The model under review builds one solid part; all positions refer to its coordinate system, in mm. Coordinates: 2 decimals unless noted, no trailing zeros. Write each loop counter-clockwise with the first axis right and the second up, starting at its lowest first coordinate (ties: lowest second). Pieces come first, ordered by that corner, then holes. Notation, with made-up numbers: (41.25, -6) - (77.25, -6) arc R17 ccw to (77.25, 12) - close; hole circle Ø4 at (0.25, 54). An arc over 180 degrees is marked (long way). Put each result on its own line as item: value.
from build123d import *

# Parameters (mm, degrees)
SKETCH_1_W          = 80
SKETCH_1_H          = 90
EXTRUDE_1_DEPTH     = 3
SKETCH_2_R          = 4.5
SKETCH_2_R_2        = 8.1
CUT_EXTRUDE_1_DEPTH = 13


with BuildPart() as part:
    # 草图1 → 凸台-拉伸1 (new, symmetric)
    with BuildSketch(Plane.XY):
        Rectangle(SKETCH_1_W, SKETCH_1_H)
    extrude(amount=EXTRUDE_1_DEPTH, both=True)

    # 草图2 → 切除-拉伸1 (cut, symmetric)
    with BuildSketch(Plane.XY):
        with Locations((-30, -30)):
            Circle(SKETCH_2_R)
        with Locations((-30, 30)):
            Circle(SKETCH_2_R)
        with Locations((30, -30)):
            Circle(SKETCH_2_R)
        with Locations((30, 30)):
            Circle(SKETCH_2_R)
        Circle(SKETCH_2_R_2)
    extrude(amount=CUT_EXTRUDE_1_DEPTH, both=True, mode=Mode.SUBTRACT)


solid = part.part
1. For pin 1 Ø5.5 at (x, y) = (30, -30) entering from +Z, flat-tipped, find the tip position at first contact; note if it passes through.
Determined:
pin 1: passes through
2. Consider section A-A on x = 30. State the section outline as (y, z) points.
Determined:
outline: (-45, -3) - (-34.5, -3) - (-34.5, 3) - (-45, 3) - close; (-25.5, -3) - (25.5, -3) - (25.5, 3) - (-25.5, 3) - close; (34.5, -3) - (45, -3) - (45, 3) - (34.5, 3) - close
3. Consider section C-C on x = 0. State the section outline as (y, z) points, plus the area to 3 significant figures.
Determined:
outline: (-45, -3) - (-8.1, -3) - (-8.1, 3) - (-45, 3) - close; (8.1, -3) - (45, -3) - (45, 3) - (8.1, 3) - close
area: 443 mm^2
4. To check wall thickness, follow probe 1 along Y at (x, z) = (-30, 0.4); probe 2 along X at (y, z) = (30, -0.8); probe 3 along Y at (x, z) = (-33, -0.95). State the ranges of each line that lie inside material, in increasing order.
Determined:
probe 1: y = -45 to -34.5, -25.5 to 25.5, 34.5 to 45
probe 2: x = -40 to -34.5, -25.5 to 25.5, 34.5 to 40
probe 3: y = -45 to -33.35, -26.65 to 26.65, 33.35 to 45
5. Consider section B-B on y = -30. State the section outline as (x, z) points, plus the area to 3 significant figures.
Determined:
outline: (-40, -3) - (-34.5, -3) - (-34.5, 3) - (-40, 3) - close; (-25.5, -3) - (25.5, -3) - (25.5, 3) - (-25.5, 3) - close; (34.5, -3) - (40, -3) - (40, 3) - (34.5, 3) - close
area: 372 mm^2
6. The part is to be moulded in two halves that separate along Y. For faces 1 (the cylindrical face through (32.08, 26.01, 0.04)), 2 (the flat face through (8.3, 0.6, 3)), 3 (the flat face through (-1, -45, 0)), say which applies: +Y half, -Y half, draft (parallel to the pull), parting line (faces both ways), or undercut.
Determined:
face 1: undercut
face 2: draft
face 3: -Y half
